from build123d import *

# Parameters (mm, degrees)
SKETCH_1_R                   = 60.5
EXTRUDE_2_DEPTH              = 12
SKETCH_3_R                   = 60.5
CUT_EXTRUDE_2_DEPTH          = 4
HOLE_WIZARD_M8_2_D           = 9
HOLE_WIZARD_M8_2_CBORE_D     = 15
HOLE_WIZARD_M8_2_CBORE_DEPTH = 9
SKETCH_11_R                  = 18
CUT_EXTRUDE_5_DEPTH          = 472.497806181
SKETCH_12_R                  = 2.5
CUT_EXTRUDE_6_DEPTH          = 472.497806181
SKETCH_13_R                  = 60.5
CUT_EXTRUDE_7_DEPTH          = 472.412962521
SKETCH_14_R                  = 5.5
CUT_EXTRUDE_8_DEPTH          = 472.497806181


with BuildPart() as part:
    # 草图1 → 凸台-拉伸2 (new body)
    with BuildSketch(Plane.XY):
        with BuildLine():
            Line((-128, 82.886556409), (384, 82.886556409))
            ThreePointArc((384, 82.886556409), (458.833147735, -25.397714839), (331.084973779, -57.113443591))
            ThreePointArc((331.084973779, -57.113443591), (318.769596292, -49.696869724), (304.627460668, -47.113443591))
            Line((304.627460668, -47.113443591), (-48.627460668, -47.113443591))
            ThreePointArc((-48.627460668, -47.113443591), (-62.769596292, -49.696869724), (-75.084973779, -57.113443591))
            ThreePointArc((-75.084973779, -57.113443591), (-202.833147735, -25.397714839), (-128, 82.886556409))
        make_face()
        with Locations((-128, 2.886556409)):
            Circle(SKETCH_1_R, mode=Mode.SUBTRACT)
        with BuildLine():
            Line((-8, 46.886556409), (92, 46.886556409))
            ThreePointArc((92, 46.886556409), (121, 17.886556409), (92, -11.113443591))
            Line((92, -11.113443591), (-8, -11.113443591))
            ThreePointArc((-8, -11.113443591), (-37, 17.886556409), (-8, 46.886556409))
        make_face(mode=Mode.SUBTRACT)
        with BuildLine():
            Line((164, 46.886556409), (264, 46.886556409))
            ThreePointArc((264, 46.886556409), (293, 17.886556409), (264, -11.113443591))
            Line((264, -11.113443591), (164, -11.113443591))
            ThreePointArc((164, -11.113443591), (135, 17.886556409), (164, 46.886556409))
        make_face(mode=Mode.SUBTRACT)
    extrude(amount=EXTRUDE_2_DEPTH)

    # 草图3 → 切除-拉伸2 (cut)
    with BuildSketch(Plane.XY):
        with Locations((384, 2.886556409)):
            Circle(SKETCH_3_R)
    extrude(amount=CUT_EXTRUDE_2_DEPTH, mode=Mode.SUBTRACT)

    # M8 六角圆柱头螺钉的柱形沉头孔2 (through all)
    with Locations(Plane(origin=(0, 0, 0), x_dir=(-1, 0, 0), z_dir=(0, 0, -1))):
        with Locations((-214, 67.886556409), (-214, -32.113443591), (-42, 67.886556409), (-42, -32.113443591)):
            CounterBoreHole(HOLE_WIZARD_M8_2_D / 2, HOLE_WIZARD_M8_2_CBORE_D / 2, HOLE_WIZARD_M8_2_CBORE_DEPTH)

    # 草图11 → 切除-拉伸5 (cut, through all)
    with BuildSketch(Plane.XY):
        with Locations((384, 2.886556409)):
            Circle(SKETCH_11_R)
    extrude(amount=CUT_EXTRUDE_5_DEPTH, mode=Mode.SUBTRACT)

    # 草图12 → 切除-拉伸6 (cut, through all)
    with BuildSketch(Plane.XY.offset(12)):
        with Locations((-78.325748622, 52.560807787)):
            Circle(SKETCH_12_R)
        with Locations((-128, 73.136556409)):
            Circle(SKETCH_12_R)
        with Locations((-57.75, 2.886556409)):
            Circle(SKETCH_12_R)
        with Locations((-78.325748622, -46.78769497)):
            Circle(SKETCH_12_R)
        with Locations((-128, -67.363443591)):
            Circle(SKETCH_12_R)
        with Locations((-177.674251378, -46.78769497)):
            Circle(SKETCH_12_R)
        with Locations((-198.25, 2.886556409)):
            Circle(SKETCH_12_R)
        with Locations((-177.674251378, 52.560807787)):
            Circle(SKETCH_12_R)
    extrude(amount=-CUT_EXTRUDE_6_DEPTH, mode=Mode.SUBTRACT)

    # 草图13 → 切除-拉伸7 (cut, through all)
    with BuildSketch(Plane(origin=(0, 0, 4), x_dir=(-1, 0, 0), z_dir=(0, 0, -1))):
        with Locations((-384, 2.886556409)):
            Circle(SKETCH_13_R)
    extrude(amount=-CUT_EXTRUDE_7_DEPTH, mode=Mode.SUBTRACT)

    # 草图14 → 切除-拉伸8 (cut, through all)
    with BuildSketch(Plane(origin=(0, 0, 0), x_dir=(-1, 0, 0), z_dir=(0, 0, -1))):
        with Locations((-384, 74.136556409)):
            Circle(SKETCH_14_R)
        with Locations((-322.29568998, 38.511556409)):
            Circle(SKETCH_14_R)
        with Locations((-322.29568998, -32.738443591)):
            Circle(SKETCH_14_R)
        with Locations((-384, -68.363443591)):
            Circle(SKETCH_14_R)
        with Locations((-445.70431002, -32.738443591)):
            Circle(SKETCH_14_R)
        with Locations((-445.70431002, 38.511556409)):
            Circle(SKETCH_14_R)
    extrude(amount=-CUT_EXTRUDE_8_DEPTH, mode=Mode.SUBTRACT)


solid = part.part
For this review, take the finished solid that the model builds, in its own axes (mm). A direction names the side the tool comes from. Coordinates: 2 decimals unless noted, no trailing zeros. Order: outer loops, then holes, each group sorted by start corner. A loop starts at its lowest first (then second) coordinate and runs counter-clockwise, first axis right, second up. Notation, with made-up numbers: (58.5, 30) - (103.5, 30) arc R17 cw to (103.5, 53) - close; hole circle Ø10 at (5.5, 30). An arc over 180 degrees is marked (long way). Answer as CSV lines item,"result". Start each with the question number.
1) To check wall thickness, follow line 1 along Y through (x, z) = (214, 3); line 2 along X through (y, z) = (-67.5, 4.25); line 3 along X through (y, z) = (51, 0.5). State the ranges of each line that lie inside material, in increasing order. Write a range as [from, to].
2) Machinability: for faces 1 (the flat face through (133, 22, 0)), 2 (the flat face through (37, 68, 9)), 3 (the cylindrical face through (135.007, 17.249, 5.916)), 4 (the flat face through (130, -47.113, 6)), which of the approach directions +Z, -Z, +X, -X, +Y, -Y give a long, thin tool a straight path to every point of the face, cutting with its end or side? Answer none if there is none.
3) Insertion check: P1, Ø3.5, axis at x = 172.5, z = 7.5, coming from the -Y side; P2, Ø2, axis at y = 28, z = 10.5, coming from the -X side; P3, Ø3, axis at y = -35.5, z = 7.5, coming from the -X side; P4, Ø4, axis at x = -128, y = -67.36, coming from the -Z side. Each pin has a flat end and moves straight along its axis. Give the tip position at first contact, or say it passes through.
4) Draft analysis for pull direction X (two halves, no side actions). For faces 5 (the flat face through (209, -32, 9)), 6 (the flat face through (209, 68, 9)), 7 (the flat face through (133, 22, 12)), state which applies: +X half, -X half, draft (parallel to the pull), parting line (faces both ways), or undercut.
5) Add section A-A (x = 8.5). State the section outline as (y, z) points.
Result:
1,line 1,"[-47.11, -39.61], [-24.61, -11.11], [46.89, 60.39], [75.39, 82.89]"
1,line 2,"[-166.02, -130.5], [-125.5, -89.98], [345.98, 378.57], [389.43, 422.02]"
1,line 3,"[-191.91, -179.63], [-175.72, -164.68], [-91.32, -80.28], [-76.37, 347.32], [420.68, 447.91]"
2,face 1,"-Z, +X, -X, +Y, -Y"
2,face 2,"-Z"
2,face 3,"+Z, -Z"
2,face 4,"+Z, -Z, -Y"
3,P1,"y = -47.11"
3,P2,"x = -204.28"
3,P3,"x = -198.99"
3,P4,"through"
4,face 5,"undercut"
4,face 6,"undercut"
4,face 7,"draft"
5,outline,"(-47.11, 0) - (-11.11, 0) - (-11.11, 12) - (-47.11, 12) - close; (46.89, 0) - (82.89, 0) - (82.89, 12) - (46.89, 12) - close"
